Read the model definition and answer for the solid it produces. Units are mm, in the model's axes. Coordinates: 2 decimals unless noted, no trailing zeros. Loops run counter-clockwise (first coordinate to the right, second up) from the corner with the lowest first, then second, coordinate; pieces in that order, holes last. Notation, with made-up numbers: (-38.75, 60.25) -> (6.25, 60.25) arc R16 ccw to (6.25, 87.25) -> close; hole circle Ø11 at (7.5, 80.25). An arc over 180 degrees is marked (long way). Answer as a JSON object with one key per item and string values. Group by question number.
1) Section A-A, the plane x = 70 is taken. Give the vertices of the cut face in (y, z), plus the area to 3 significant figures.
2) Section C-C, the plane y = 69.5 is taken. Give the vertices of the cut face in (x, z).
3) Consider probe 1 along Z at (x, y) = (-34, 65.5); probe 2 along Y at (x, z) = (59, 15.75); probe 3 along Y at (x, z) = (-38.5, 16). Determine where each line is inside the solid, lowest interval first. Write a range as [from, to].
4) Section B-B, the plane z = 17.25 is taken. Give the vertices of the cut face in (x, y), plus the area to 3 significant figures.
from build123d import *

# Parameters (mm, degrees)
SKETCH_1_W      = 180
SKETCH_1_H      = 75
EXTRUDE_1_DEPTH = 20
CHAMFER_2_SIZE  = 10


with BuildPart() as part:
    # 草图1 → 凸台-拉伸1 (new body)
    with BuildSketch(Plane.XY):
        with Locations((0, 37.5)):
            Rectangle(SKETCH_1_W, SKETCH_1_H)
    extrude(amount=EXTRUDE_1_DEPTH)

    # 倒角2
    chamfer_2_edges = [part.edges().sort_by_distance(p)[0] for p in [
        (0, 75, 20),
    ]]
    chamfer(chamfer_2_edges, length=CHAMFER_2_SIZE)


solid = part.part
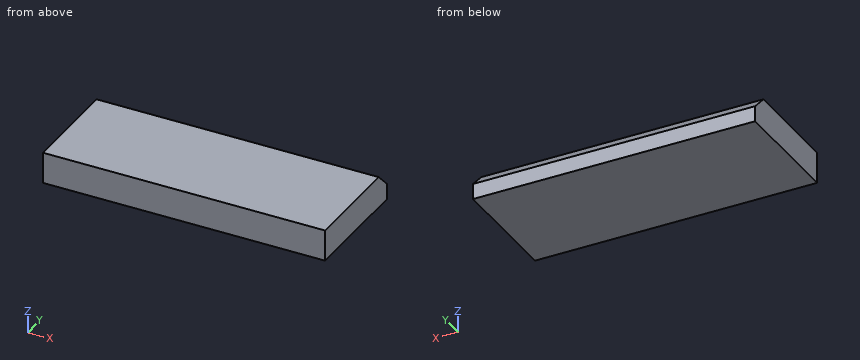
Determined:
{
 "1": {"outline": "(0, 0) -> (75, 0) -> (75, 10) -> (65, 20) -> (0, 20) -> close", "area": "1,450 mm²"},
 "2": {"outline": "(-90, 0) -> (90, 0) -> (90, 15.5) -> (-90, 15.5) -> close"},
 "3": {"probe 1": "[0, 19.5]", "probe 2": "[0, 69.25]", "probe 3": "[0, 69]"},
 "4": {"outline": "(-90, 0) -> (90, 0) -> (90, 67.75) -> (-90, 67.75) -> close", "area": "12,200 mm²"}
}
